```python
from build123d import *

# Parameters (mm, degrees)
BOSS_EXTRUDE1_DEPTH = 5.4
M12_TAPPED_HOLE1_D  = 10.2


with BuildPart() as part:
    # Sketch1 → Boss-Extrude1 (new, symmetric)
    with BuildSketch(Plane.XY):
        Polygon((8.65, -4.994079828), (8.65, 4.994079828), (0, 9.988159657), (-8.65, 4.994079828), (-8.65, -4.994079828), (0, -9.988159657), align=None)
    extrude(amount=BOSS_EXTRUDE1_DEPTH, both=True)

    # M12 Tapped Hole1 (through all)
    with Locations(Plane.XY.offset(5.4)):
        with Locations((0, 0)):
            Hole(M12_TAPPED_HOLE1_D / 2)


solid = part.part
```
The listing builds one solid part. Answer for the finished solid, in the listing's coordinates (mm). Round coordinates to 2 decimals unless told otherwise and drop trailing zeros. Loops run counter-clockwise (first coordinate to the right, second up) from the corner with the lowest first, then second, coordinate; pieces in that order, holes last. Notation, with made-up numbers: (57, -7.5) -> (81, -7.5) arc R15 cw to (81, 6.5) -> close; hole circle Ø9 at (88, -22). An arc over 180 degrees is marked (long way). Use one line per item in the form item = value.
1. For a pull along Y with two mould halves and no side action, classify faces 1 (the flat face through (4.386, 7.456, 0.076)), 2 (the flat face through (8.65, 0, 0)), 3 (the cylindrical face through (-2.4, -4.5, -0.1)) as released by +Y, released by -Y, zero draft, split by the parting line, or undercut.
Answer key:
face_1 = released by +Y
face_2 = zero draft
face_3 = undercut
2. The part is cut by section B-B on y = 0. Determine the outline of the cut face in (x, z).
Answer key:
outline = (-8.65, -5.4) -> (-5.1, -5.4) -> (-5.1, 5.4) -> (-8.65, 5.4) -> close; (5.1, -5.4) -> (8.65, -5.4) -> (8.65, 5.4) -> (5.1, 5.4) -> close
3. The part is cut by section A-A on z = 0. Determine the outline of the cut face in (x, y), and give its area (3 significant figures).
Answer key:
outline = (-8.65, -4.99) -> (0, -9.99) -> (8.65, -4.99) -> (8.65, 4.99) -> (0, 9.99) -> (-8.65, 4.99) -> close; hole circle Ø10.2 at (0, 0)
area = 177 mm²
4. Find the intervals of material crossed by probe 1 along X at (y, z) = (-2, 0.25); probe 2 along X at (y, z) = (-1.5, 4.5); probe 3 along Y at (x, z) = (-4, 1.75), in increasing order. Write a range as [from, to].
Answer key:
probe_1 = [-8.65, -4.69], [4.69, 8.65]
probe_2 = [-8.65, -4.87], [4.87, 8.65]
probe_3 = [-7.68, -3.16], [3.16, 7.68]
5. Flat-ended cylindrical pins translate along their axes: pin 1 Ø1 at (x, z) = (-3, -3.5) entering from -Y; pin 2 Ø3 at (x, z) = (-3.5, 2) entering from -Y; pin 3 Ø1 at (x, z) = (3.5, -2) entering from -Y; pin 4 Ø8 at (x, y) = (0, 0) entering from +Z. Find the tip coordinate at first contact, or state that the pin passes through.
Answer key:
pin_1 = -8.54
pin_2 = -8.83
pin_3 = -8.26
pin_4 = through
6. The part is cut by section D-D on x = -7.5. Determine the outline of the cut face in (y, z), and give its area (3 significant figures).
Answer key:
outline = (-5.66, -5.4) -> (5.66, -5.4) -> (5.66, 5.4) -> (-5.66, 5.4) -> close
area = 122 mm²
7. The part is cut by section C-C on x = 3. Determine the outline of the cut face in (y, z), and give its area (3 significant figures).
Answer key:
outline = (-8.26, -5.4) -> (-4.12, -5.4) -> (-4.12, 5.4) -> (-8.26, 5.4) -> close; (4.12, -5.4) -> (8.26, -5.4) -> (8.26, 5.4) -> (4.12, 5.4) -> close
area = 89.2 mm²
